Could you check a few things on this drawing? It's one solid part, dimensions in mm from its lowest x, y, z. A direction names the side the tool comes from. Give positions to 0.01 mm unless a question says otherwise; leave off trailing zeros. Write each loop counter-clockwise with the first axis right and the second up, starting at its lowest first coordinate (ties: lowest second). Pieces come first, ordered by that corner, then holes. Notation, with made-up numbers: (71, 45.5) -> (98, 45.5) arc R15 ccw to (98, 51.5) -> close; hole circle Ø2 at (-35.75, -2.5). An arc over 180 degrees is marked (long way). Use CSV: the item, a comma, the result in double quotes. Start each with the question number.
(1) For pin 1 Ø12 at (y, z) = (32, 11.5) entering from +X; pin 2 Ø4 at (y, z) = (17, 21.5) entering from -X; pin 3 Ø6 at (y, z) = (23, 14) entering from -X, each with a flat end and sliding along its axis, tell me the tip position at first contact or that it passes through.
(2) Suppose I cut it at B-B on x = 24. List the corners of the cut face in (y, z) for me, plus the area to 3 significant figures.
(3) I need wall thicknesses on L1, parallel to Z at x = 24, y = 24.5; L2, parallel to Y at x = 24, z = 43.5. Which ranges of each line are inside material? Lowest first, please. Write a range as [from, to].
(4) Which directions (+Z, -Z, +X, -X, +Y, -Y) give clear straight access to the entire face, cutting with the end or side of a thin tool? Please do the marked faces 4 and 5.
(5) Suppose I cut it at C-C on y = 3.5. List the corners of the cut face in (x, z) for me.
(6) If we mould it in two halves opening along Y, with no side actions, what happens to the marked faces 1, 2 and 3? For each: pulls with the +Y half, pulls with the -Y half, needs draft (parallel to the pull), parting line crosses it, or undercut.
(7) Suppose I cut it at A-A on z = 24. List the corners of the cut face in (x, y) for me.
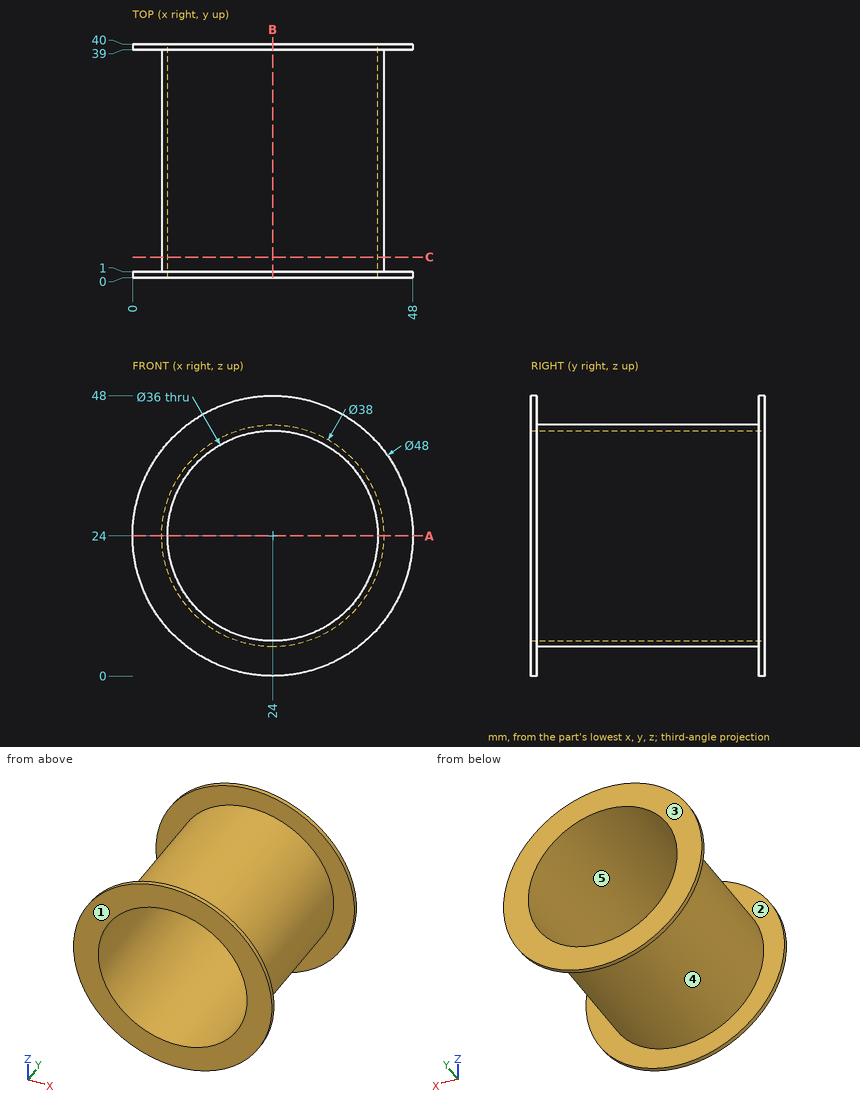
Geometry says:
1,pin 1,"x = 41.85"
1,pin 2,"x = 5.01"
1,pin 3,"x = 6.34"
2,outline,"(0, 0) -> (1, 0) -> (1, 5) -> (39, 5) -> (39, 0) -> (40, 0) -> (40, 6) -> (0, 6) -> close; (0, 42) -> (40, 42) -> (40, 48) -> (39, 48) -> (39, 43) -> (1, 43) -> (1, 48) -> (0, 48) -> close"
2,area,"100 mm²"
3,L1,"[5, 6], [42, 43]"
3,L2,"[0, 1], [39, 40]"
4,face 4,"none"
4,face 5,"+Y, -Y"
5,outline,"circle Ø38 at (24, 24); hole circle Ø36 at (24, 24)"
6,face 1,"pulls with the -Y half"
6,face 2,"undercut"
6,face 3,"pulls with the +Y half"
7,outline,"(0, 0) -> (6, 0) -> (6, 40) -> (0, 40) -> (0, 39) -> (5, 39) -> (5, 1) -> (0, 1) -> close; (42, 0) -> (48, 0) -> (48, 1) -> (43, 1) -> (43, 39) -> (48, 39) -> (48, 40) -> (42, 40) -> close"
